from build123d import *

# Parameters (mm, degrees)
BOSS_EXTRUDE1_DEPTH    = 8
SKETCH6_R              = 5
SKETCH6_W              = 18
SKETCH6_H              = 25
CUT_EXTRUDE1_DEPTH     = 39.807215824
M4_TAPPED_HOLE1_REACH  = 58.471
M4_TAPPED_HOLE1_BORE_R = 1.65
M3_TAPPED_HOLE1_D      = 2.5
SKETCH13_W             = 32
SKETCH13_H             = 50
CUT_EXTRUDE2_DEPTH     = 1
SKETCH14_W             = 20
SKETCH14_H             = 5
CUT_EXTRUDE3_DEPTH     = 39.80721593
CHAMFER1_SIZE          = 3
FILLET1_R              = 3
CHAMFER3_SIZE          = 1
CHAMFER4_SIZE          = 0.5
FILLET2_R              = 1


with BuildPart() as part:
    # Sketch1 → Boss-Extrude1 (new, symmetric)
    with BuildSketch(Plane.XY):
        Polygon((-25, -10), (-25, -25), (25, -25), (25, -10), (25, 25), (-25, 25), align=None)
    extrude(amount=BOSS_EXTRUDE1_DEPTH, both=True)

    # Sketch6 → Cut-Extrude1 (cut, through all)
    with BuildSketch(Plane.XY.offset(8)):
        with Locations((-17.5, 15)):
            Circle(SKETCH6_R)
        with Locations((17.5, 15)):
            Circle(SKETCH6_R)
        with Locations((16, -4.5)):
            Rectangle(SKETCH6_W, SKETCH6_H)
        with Locations((-16, -4.5)):
            Rectangle(SKETCH6_W, SKETCH6_H)
    extrude(amount=-CUT_EXTRUDE1_DEPTH, mode=Mode.SUBTRACT)

    # M4 Tapped Hole1 bore → M4 Tapped Hole1 (cut, up to next)
    with BuildSketch(Plane(origin=(0, 25, 0), x_dir=(1, 0, 0), z_dir=(0, 1, 0)), mode=Mode.PRIVATE) as m4_tapped_hole1_sk1:
        with Locations((-17.5, 0)):
            Circle(M4_TAPPED_HOLE1_BORE_R)
    m4_tapped_hole1_tool1 = extrude(m4_tapped_hole1_sk1.sketch, amount=-M4_TAPPED_HOLE1_REACH, mode=Mode.PRIVATE) & part.part
    # M4 Tapped Hole1 bore → M4 Tapped Hole1 (cut, up to next)
    with BuildSketch(Plane(origin=(0, 25, 0), x_dir=(1, 0, 0), z_dir=(0, 1, 0)), mode=Mode.PRIVATE) as m4_tapped_hole1_sk2:
        with Locations((17.5, 0)):
            Circle(M4_TAPPED_HOLE1_BORE_R)
    m4_tapped_hole1_tool2 = extrude(m4_tapped_hole1_sk2.sketch, amount=-M4_TAPPED_HOLE1_REACH, mode=Mode.PRIVATE) & part.part
    add(m4_tapped_hole1_tool1.solids().sort_by_distance((-17.5, 25, 0))[0], mode=Mode.SUBTRACT)
    add(m4_tapped_hole1_tool2.solids().sort_by_distance((17.5, 25, 0))[0], mode=Mode.SUBTRACT)

    # M3 Tapped Hole1 (through all)
    with Locations(Plane.XY.offset(8)):
        with Locations((0, -19), (0, 16)):
            Hole(M3_TAPPED_HOLE1_D / 2)

    # Sketch13 → Cut-Extrude2 (cut)
    with BuildSketch(Plane.XY.offset(-8)):
        Rectangle(SKETCH13_W, SKETCH13_H)
    extrude(amount=CUT_EXTRUDE2_DEPTH, mode=Mode.SUBTRACT)

    # Sketch14 → Cut-Extrude3 (cut, through all)
    with BuildSketch(Plane.XY.offset(8)):
        with Locations((0, 22.5)):
            Rectangle(SKETCH14_W, SKETCH14_H)
    extrude(amount=-CUT_EXTRUDE3_DEPTH, mode=Mode.SUBTRACT)

    # Chamfer1
    chamfer1_edges = [part.edges().sort_by_distance(p)[0] for p in [
        (-25, 25, 0),
        (25, 25, 0),
    ]]
    chamfer(chamfer1_edges, length=CHAMFER1_SIZE)

    # Fillet1
    fillet1_edges = [part.edges().sort_by_distance(p)[0] for p in [
        (-7, -17, 0.5),
        (-7, 8, 0.5),
        (7, -17, 0.5),
        (7, 8, 0.5),
    ]]
    fillet(fillet1_edges, radius=FILLET1_R)

    # Chamfer3
    chamfer3_edges = [part.edges().sort_by_distance(p)[0] for p in [
        (-10, 25, 0.5),
        (10, 25, 0.5),
        (25, 8, 0),
        (25, -17, 0),
        (-25, -17, 0),
        (-25, 8, 0),
    ]]
    chamfer(chamfer3_edges, length=CHAMFER3_SIZE)

    # Chamfer4
    chamfer4_edges = [part.edges().sort_by_distance(p)[0] for p in [
        (-22.5, 15, -8),
        (-22.5, 15, 8),
        (12.5, 15, 8),
        (20.458039892, 19.031128874, -8),
    ]]
    chamfer(chamfer4_edges, length=CHAMFER4_SIZE)

    # Fillet2
    fillet2_edges = [part.edges().sort_by_distance(p)[0] for p in [
        (-10, 20, 0.5),
        (10, 20, 0.5),
    ]]
    fillet(fillet2_edges, radius=FILLET2_R)


solid = part.part
Here's how the part is built. I have some questions about the finished solid (model axes, mm). A direction names the side the tool comes from. Coordinates: 2 decimals unless noted, no trailing zeros. Order: outer loops, then holes, each group sorted by start corner. A loop starts at its lowest first (then second) coordinate and runs counter-clockwise, first axis right, second up.
Item 1: If we section it at A-A on x = -17.5: List the corners of the cut face in (y, z) for me.
Result sheet:
outline: (-25, -8) - (-17, -8) - (-17, 8) - (-25, 8) - close; (8, -8) - (9.5, -8) - (10, -7.5) - (10, 7.5) - (9.5, 8) - (8, 8) - close; (20, -7.5) - (20.5, -8) - (25, -8) - (25, -1.65) - (20, -1.65) - close; (20, 1.65) - (25, 1.65) - (25, 8) - (20.5, 8) - (20, 7.5) - close
Item 2: For P1, Ø3, axis at y = -10, z = -2.5, coming from the +X side; P2, Ø0.8, axis at y = 22.5, z = -7.5, coming from the +X side; P3, Ø5, axis at y = -10.5, z = 2.5, coming from the -X side, each with a flat end and sliding along its axis, tell me the tip position at first contact or that it passes through.
Result sheet:
P1: stops at x = 7
P2: stops at x = 24.9
P3: stops at x = -7
Item 3: For faces 1 (the face through (19.074, 22.394, -0.496)), 2 (the face through (7.86, 7.1, 0.39)), 3 (the face through (0, 20, 1)), which set-ups out of +Z, -Z, +X, -X, +Y, -Y let a thin tool reach every point of the face, with its end or its side?
Result sheet:
face 1: +Y
face 2: +Z, -Z, +X
face 3: +Z, -Z, +Y
Item 4: If we section it at B-B on y = -19: List the corners of the cut face in (x, z) for me.
Result sheet:
outline: (-25, -8) - (-16, -8) - (-16, -7) - (-1.25, -7) - (-1.25, 8) - (-25, 8) - close; (1.25, -7) - (16, -7) - (16, -8) - (25, -8) - (25, 8) - (1.25, 8) - close
Item 5: If we section it at C-C on x = 0: List the corners of the cut face in (y, z) for me, plus the area to 3 significant figures.
Result sheet:
outline: (-25, -7) - (-20.25, -7) - (-20.25, 8) - (-25, 8) - close; (-17.75, -7) - (14.75, -7) - (14.75, 8) - (-17.75, 8) - close; (17.25, -7) - (20, -7) - (20, 8) - (17.25, 8) - close
area: 600 mm2
Item 6: If we mould it in two halves opening along Y, with no side actions, what happens to faces 4 (the face through (16.42, 10.12, 0.11)), 5 (the face through (-17, -17, 0)), 6 (the face through (-15, 25, 0)), 7 (the face through (25, 15, 0))? For each: +Y half, -Y half, draft (parallel to the pull), parting line (faces both ways), or undercut.
Result sheet:
face 4: undercut
face 5: undercut
face 6: +Y half
face 7: draft
Item 7: If we section it at D-D on z = 6: State how many separate pieces and enclosed holes the cut face has, plus the area to 3 significant figures.
Result sheet:
separate pieces: 1
enclosed holes: 4
area: 1,330 mm2
Item 8: I need wall thicknesses on line 1 (Y direction, x = 0, z = 4); line 2 (Y direction, x = 17.5, z = 5.5); line 3 (X direction, y = 21.2, z = 0). Which ranges of each line are inside material? Lowest first, please.
Result sheet:
line 1: y = -25 to -20.25, -17.75 to 14.75, 17.25 to 20
line 2: y = -25 to -17, 8 to 10, 20 to 25
line 3: x = -25 to -19.15, -15.85 to -10, 10 to 15.85, 19.15 to 25
